Answer from the drawing. Dimensions are ordinates in mm from the lowest x, y and z of the part. A direction names the side the tool comes from. Give positions to 0.01 mm unless a question says otherwise; leave off trailing zeros. Loops run counter-clockwise (first coordinate to the right, second up) from the corner with the lowest first, then second, coordinate; pieces in that order, holes last. Notation, with made-up numbers: (52, -10.5) -> (100, -10.5) arc R19 ccw to (100, 22.5) -> close; hole circle Ø2 at (46.5, 42). An arc over 180 degrees is marked (long way). Write each question's results on one line, items separated by ' | '. Start each with the question number.
Item 1: Which of the six approach directions +Z, -Z, +X, -X, +Y, -Y give full straight-line access (tool end or side, diameter ignored) to the marked faces 1 and 2?
Item 2: Section C-C on y = 62 is taken. Write down the section's boundary in (x, z), and give its area (3 significant figures).
Item 3: Find the intervals of material crossed by line 1 (Z direction, x = 16.5, y = 59.5); line 2 (Y direction, x = 20, z = 17.75), in increasing order.
Item 4: Section A-A on x = 9.5 is taken. Write down the section's boundary in (y, z), and give its area (3 significant figures).
Item 5: Section B-B on z = 21 is taken. Write down the section's boundary in (x, y), and give its area (3 significant figures).
Item 6: Each of these flat-tipped pins is pushed along its axis until it touches: P1, Ø11.5, axis at x = 25, y = 21, coming from the +Z side; P2, Ø4, axis at x = 30.5, z = 19.5, coming from the -Y side; P3, Ø4, axis at y = 44, z = 9.5, coming from the +X side. Where does it stop, or does it pass through?
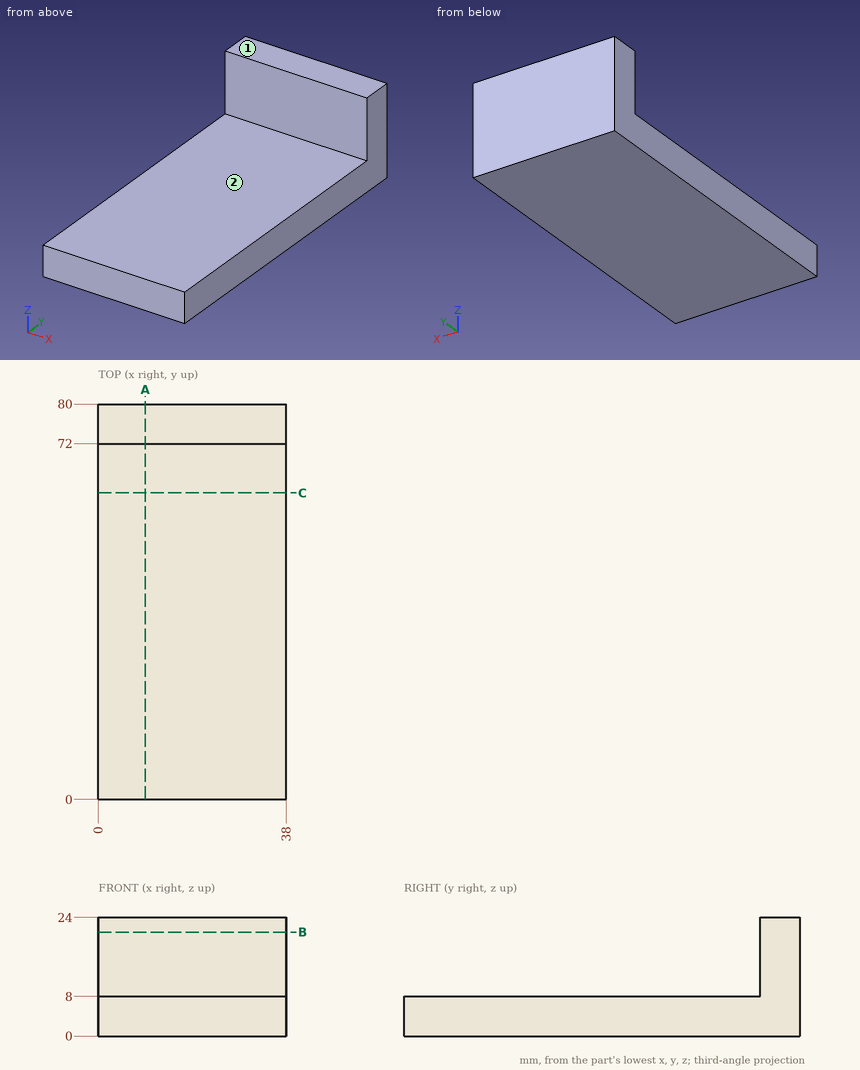
Findings:
1) face 1: +Z, +X, -X, +Y, -Y | face 2: +Z, +X, -X, -Y
2) outline: (0, 0) -> (38, 0) -> (38, 8) -> (0, 8) -> close | area: 304 mm2
3) line 1: 0 to 8 | line 2: 72 to 80
4) outline: (0, 0) -> (80, 0) -> (80, 24) -> (72, 24) -> (72, 8) -> (0, 8) -> close | area: 768 mm2
5) outline: (0, 72) -> (38, 72) -> (38, 80) -> (0, 80) -> close | area: 304 mm2
6) P1: z = 8 | P2: y = 72 | P3: x = 38
